Design review of the part built by this model. Coordinates are the model's own, in mm. Give positions to 0.01 mm unless a question says otherwise; leave off trailing zeros. Loops run counter-clockwise (first coordinate to the right, second up) from the corner with the lowest first, then second, coordinate; pieces in that order, holes last. Notation, with made-up numbers: (-11.5, 61.25) - (35.5, 61.25) arc R7 ccw to (35.5, 72.25) - close; hole circle Ø10 at (84.5, 75). An arc over 180 degrees is marked (long way). Write each question's results on one line, items separated by ' | '.
```python
from build123d import *

# Parameters (mm, degrees)
SKETCH_1_W          = 380
SKETCH_1_H          = 320
EXTRUDE_1_DEPTH     = 1.5
SKETCH_2_R          = 6
CUT_EXTRUDE_1_DEPTH = 11.5


with BuildPart() as part:
    # 草图1 → 凸台-拉伸1 (new, symmetric)
    with BuildSketch(Plane.XY):
        Rectangle(SKETCH_1_W, SKETCH_1_H)
    extrude(amount=EXTRUDE_1_DEPTH, both=True)

    # 草图2 → 切除-拉伸1 (cut, symmetric)
    with BuildSketch(Plane.XY):
        with Locations((130, -100)):
            Circle(SKETCH_2_R)
    extrude(amount=CUT_EXTRUDE_1_DEPTH, both=True, mode=Mode.SUBTRACT)


solid = part.part
```
Item 1: Wall thickness on probe 1 along Y at (x, z) = (130, 0.85); probe 2 along X at (y, z) = (-101, -0.25); probe 3 along X at (y, z) = (-96.5, 0.6): over which ranges is each line inside the solid? List them lowest first.
Output values:
probe 1: y = -160 to -106, -94 to 160 | probe 2: x = -190 to 124.08, 135.92 to 190 | probe 3: x = -190 to 125.13, 134.87 to 190
Item 2: We need section B-B on y = -100. Give the boundary of the cut face in (x, z).
Output values:
outline: (-190, -1.5) - (124, -1.5) - (124, 1.5) - (-190, 1.5) - close; (136, -1.5) - (190, -1.5) - (190, 1.5) - (136, 1.5) - close
Item 3: Draft analysis for pull direction X (two halves, no side actions). For faces 1 (the face through (-3, 2, -1.5)), 2 (the face through (125.58, -95.94, 0.02)), state which applies: +X half, -X half, draft (parallel to the pull), parting line (faces both ways), or undercut.
Output values:
face 1: draft | face 2: undercut
Item 4: We need section A-A on x = 130. Give the boundary of the cut face in (y, z).
Output values:
outline: (-160, -1.5) - (-106, -1.5) - (-106, 1.5) - (-160, 1.5) - close; (-94, -1.5) - (160, -1.5) - (160, 1.5) - (-94, 1.5) - close
Item 5: Clearance check with a flat-ended pin moving along its axis: P1, Ø9.5, axis at x = 130, y = -100, coming from the -Z side. State where the tip first meets the part, or that it passes through.
Output values:
P1: passes through
